Source: three-view drawing plus pictorial views. Frame: mm from the lowest corner of the part. A direction names the side the tool comes from. Give positions to 0.01 mm unless a question says otherwise; leave off trailing zeros. Loops run counter-clockwise (first coordinate to the right, second up) from the corner with the lowest first, then second, coordinate; pieces in that order, holes last. Notation, with made-up numbers: M 73.25,-25.75 L 95.25,-25.75 A5 cw 95.25,-17.75 Z; hole C -20.75,15.25 d6. An arc over 180 degrees is marked long. Write item = value, one per line.
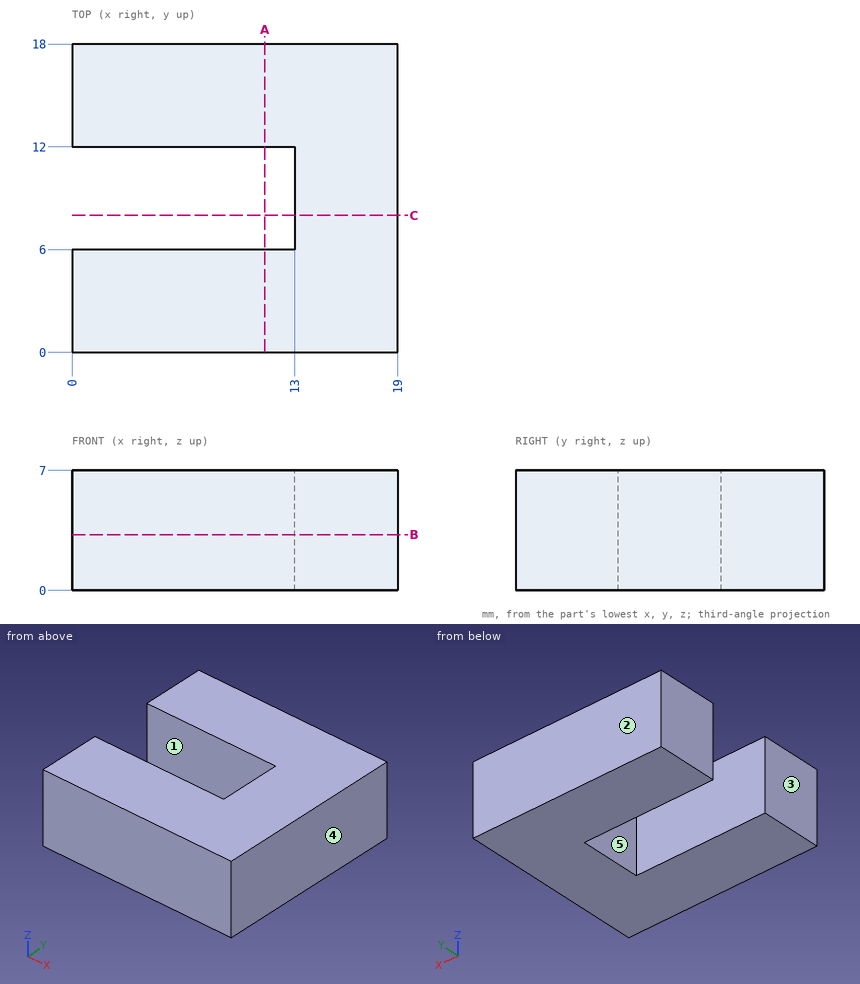
1. Pull-direction query (Y, two-part tool) for the marked faces 1, 2 and 3; classes: +Y half, -Y half, draft (parallel to the pull), parting line (faces both ways), or undercut.
Derived:
face_1 = undercut
face_2 = +Y half
face_3 = draft
2. Cut plane C-C, the plane y = 8. Return the cut outline in (x, z), then the cut area to 3 significant figures.
Derived:
outline = M 13,0 L 19,0 L 19,7 L 13,7 Z
area = 42.0 mm²
3. Material intervals for probe 1 along Y at (x, z) = (11.75, 1.75); probe 2 along X at (y, z) = (10, 5.5), sorted ascending. Write a range as from..to.
Derived:
probe_1 = 0..6, 12..18
probe_2 = 13..19
4. Reachability of the marked faces 4 and 5 from +Z, -Z, +X, -X, +Y, -Y: full face, straight path, thin tool, end or side. Return the list, or none.
Derived:
face_4 = +Z, -Z, +X, +Y, -Y
face_5 = +Z, -Z, -X
5. First-contact query: pin 1 Ø2 at (y, z) = (9.5, 4) entering from -X. Flat tip, straight axial feed; report the tip coordinate or a pass-through.
Derived:
pin_1 = 13
6. Cut plane A-A, the plane x = 11.25. Return the cut outline in (y, z), then the cut area to 3 significant figures.
Derived:
outline = M 0,0 L 6,0 L 6,7 L 0,7 Z; M 12,0 L 18,0 L 18,7 L 12,7 Z
area = 84.0 mm²
7. Cut plane B-B, the plane z = 3.25. Return the cut outline in (x, y), then the cut area to 3 significant figures.
Derived:
outline = M 0,0 L 19,0 L 19,18 L 0,18 L 0,12 L 13,12 L 13,6 L 0,6 Z
area = 264 mm²
